Part model, mm, in its own coordinate system. Face numbers are marked on the shaded views. A direction names the side the tool comes from. Give positions to 0.01 mm unless a question says otherwise; leave off trailing zeros. Write each loop counter-clockwise with the first axis right and the second up, starting at its lowest first coordinate (ties: lowest second). Pieces come first, ordered by that corner, then holes.
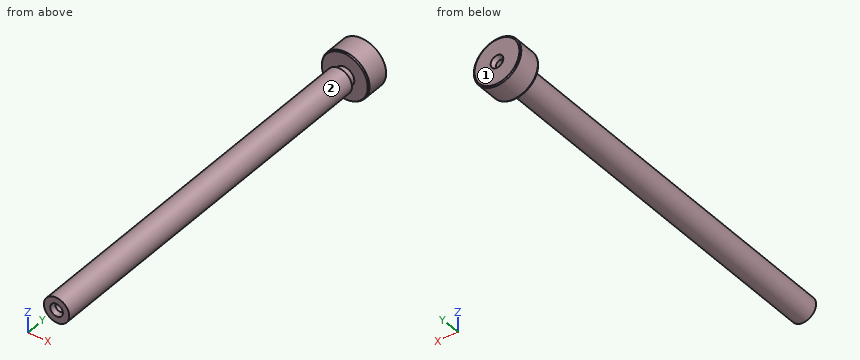
from build123d import *
from OCP.BRepFilletAPI import BRepFilletAPI_MakeChamfer

# Parameters (mm, degrees)
F_5_0MM_DOWEL_HOLE1_D     = 5
F_5_0MM_DOWEL_HOLE1_DEPTH = 5
F_5_0MM_DOWEL_HOLE1_TIP   = 1.502151548
CHAMFER1_SIZE             = 1.5
CHAMFER1_SIZE2            = 2.496419224
CHAMFER2_SIZE             = 0.5
CHAMFER2_SIZE2            = 0.832139741
F_5_0MM_DOWEL_HOLE2_D     = 5
F_5_0MM_DOWEL_HOLE2_DEPTH = 5
F_5_0MM_DOWEL_HOLE2_TIP   = 1.502151548
CHAMFER3_SIZE             = 1.5
CHAMFER3_SIZE2            = 2.496419224


with BuildPart() as part:
    # Sketch1 → Revolve1 (revolve)
    with BuildSketch(Plane.XY, mode=Mode.PRIVATE) as revolve1_sk:
        Polygon((0, 252), (15, 252), (15, 237), (6, 237), (6, 233), (8, 233), (8, 0), (0, 0), align=None)
    revolve(revolve1_sk.sketch.rotate(Axis((0, 252, 0), (0, -1, 0)), 180), axis=Axis((0, 252, 0), (0, -1, 0)))

    # Ø5.0mm Dowel Hole1
    with Locations(Plane(origin=(0, 0, 0), x_dir=(-1, 0, 0), z_dir=(0, -1, 0))):
        with Locations((0, 0), (163.193456079, -92.802944279)):
            Hole(F_5_0MM_DOWEL_HOLE1_D / 2, depth=F_5_0MM_DOWEL_HOLE1_DEPTH)
            with Locations((0, 0, -(F_5_0MM_DOWEL_HOLE1_DEPTH + F_5_0MM_DOWEL_HOLE1_TIP / 2))):  # 118° drill point
                Cone(0, F_5_0MM_DOWEL_HOLE1_D / 2, F_5_0MM_DOWEL_HOLE1_TIP, mode=Mode.SUBTRACT)

    # Chamfer1
    chamfer1_edges = [part.edges().sort_by_distance(p)[0] for p in [
        (-2.5, 0, 0),
    ]]
    chamfer1_side = [part.faces().sort_by_distance(p)[0] for p in [
        (7.77372583, 0, 0),
    ]]
    chamfer(chamfer1_edges, length=CHAMFER1_SIZE, length2=CHAMFER1_SIZE2, reference=chamfer1_side[0])

    # Chamfer2: one chamfer whose edges measure the first distance from different faces: ONE call of the kernel's chamfer builder (chamfer() names one face for all edges)
    chamfer2_edges_1 = [part.edges().sort_by_distance(p)[0] for p in [
        (15, 237, 0),
    ]]
    chamfer2_side_1 = [part.faces().sort_by_distance(p)[0] for p in [
        (14.575735931, 237, 0),
    ]]
    chamfer2_edges_2 = [part.edges().sort_by_distance(p)[0] for p in [
        (15, 252, 0),
    ]]
    chamfer2_side_2 = [part.faces().sort_by_distance(p)[0] for p in [
        (15, 244.5, 0),
    ]]
    chamfer2_edges_3 = [part.edges().sort_by_distance(p)[0] for p in [
        (8, 233, 0),
    ]]
    chamfer2_side_3 = [part.faces().sort_by_distance(p)[0] for p in [
        (8, 116.5, 0),
    ]]
    chamfer2 = BRepFilletAPI_MakeChamfer(part.part.solid().wrapped)
    for e in chamfer2_edges_1:
        chamfer2.Add(CHAMFER2_SIZE, CHAMFER2_SIZE2, e.wrapped, chamfer2_side_1[0].wrapped)  # the first distance lies on this face
    for e in chamfer2_edges_2:
        chamfer2.Add(CHAMFER2_SIZE, CHAMFER2_SIZE2, e.wrapped, chamfer2_side_2[0].wrapped)  # the first distance lies on this face
    for e in chamfer2_edges_3:
        chamfer2.Add(CHAMFER2_SIZE, CHAMFER2_SIZE2, e.wrapped, chamfer2_side_3[0].wrapped)  # the first distance lies on this face
    add(Compound.cast(chamfer2.Shape()), mode=Mode.REPLACE)

    # Ø5.0mm Dowel Hole2
    with Locations(Plane(origin=(0, 252, 0), x_dir=(1, 0, 0), z_dir=(0, 1, 0))):
        with Locations((0, 0)):
            Hole(F_5_0MM_DOWEL_HOLE2_D / 2, depth=F_5_0MM_DOWEL_HOLE2_DEPTH)
            with Locations((0, 0, -(F_5_0MM_DOWEL_HOLE2_DEPTH + F_5_0MM_DOWEL_HOLE2_TIP / 2))):  # 118° drill point
                Cone(0, F_5_0MM_DOWEL_HOLE2_D / 2, F_5_0MM_DOWEL_HOLE2_TIP, mode=Mode.SUBTRACT)

    # Chamfer3
    chamfer3_edges = [part.edges().sort_by_distance(p)[0] for p in [
        (2.5, 252, 0),
    ]]
    chamfer3_side = [part.faces().sort_by_distance(p)[0] for p in [
        (13.767132656, 252, 0),
    ]]
    chamfer(chamfer3_edges, length=CHAMFER3_SIZE, length2=CHAMFER3_SIZE2, reference=chamfer3_side[0])


solid = part.part
1) Drill centre lines: L1, parallel to Z at x = 0, y = 4.45; L2, parallel to Z at x = 0, y = 248.95; L3, parallel to Y at x = 2.75, z = 13.5. Where is each one in solid material? Low to high.
Check result:
L1: z = -8 to -2.5, 2.5 to 8
L2: z = -15 to -2.5, 2.5 to 15
L3: y = 237 to 252
2) 3-axis set-ups, long thin cutter, end or side, ignore diameter. For the marked faces 1 and 2: which of +Z, -Z, +X, -X, +Y, -Y reach the whole face in a straight line?
Check result:
face 1: +Z, -Z, +X, -X, +Y
face 2: -Y
3) Saw through at A-A (y = 31). Write the cut outline in (x, z).
Check result:
outline: circle Ø16 at (0, 0)
4) Flat gauge pins, fed straight in: P1, Ø3, axis at x = 0, z = 0, coming from the -Y side; P2, Ø4, axis at x = 0, z = 0, coming from the -Y side; P3, Ø1, axis at x = 2.5, y = 70.5, coming from the +Z side. Where does each tip first touch, or does it go through?
Check result:
P1: stops at y = 5.6
P2: stops at y = 5.3
P3: stops at z = 7.75
